For this review, take the finished solid that the model builds, in its own axes (mm). Face numbers are marked on the shaded views. A direction names the side the tool comes from. Give positions to 0.01 mm unless a question says otherwise; leave off trailing zeros. Loops run counter-clockwise (first coordinate to the right, second up) from the corner with the lowest first, then second, coordinate; pieces in that order, holes last. Notation, with made-up numbers: (-9.5, -37.5) - (0.5, -37.5) arc R23 ccw to (0.5, -6.5) - close; hole circle Ø9 at (11.5, 10.25). An arc over 180 degrees is marked (long way). Answer as CSV lines item,"result".
from build123d import *

# Parameters (mm, degrees)
SKETCH3_W           = 52
SKETCH3_H           = 52
BOSS_EXTRUDE1_DEPTH = 10
SKETCH4_R           = 2
CUT_EXTRUDE1_DEPTH  = 10
SKETCH5_R           = 25
CUT_EXTRUDE2_DEPTH  = 3
SKETCH6_R           = 16
CUT_EXTRUDE3_DEPTH  = 38.429934544
SKETCH8_W           = 21.53152206
SKETCH8_H           = 52
BOSS_EXTRUDE2_DEPTH = 52
SKETCH9_R           = 20
CUT_EXTRUDE4_DEPTH  = 21.53152206
BOSS_EXTRUDE3_DEPTH = 52
SKETCH11_R          = 20
CUT_EXTRUDE5_DEPTH  = 52
SKETCH12_W          = 34.659031173
SKETCH12_H          = 60
CUT_EXTRUDE6_DEPTH  = 10


with BuildPart() as part:
    # Sketch3 → Boss-Extrude1 (new body)
    with BuildSketch(Plane.XY):
        Rectangle(SKETCH3_W, SKETCH3_H)
    extrude(amount=BOSS_EXTRUDE1_DEPTH)

    # Sketch4 → Cut-Extrude1 (cut)
    with BuildSketch(Plane(origin=(0, 0, 0), x_dir=(-1, 0, 0), z_dir=(0, 0, -1))):
        with Locations((-21, 21)):
            Circle(SKETCH4_R)
        with Locations(Location((21, 21, 0), (0, 0, 180))):
            Circle(SKETCH4_R)
        with Locations((21, -21)):
            Circle(SKETCH4_R)
        with Locations(Location((-21, -21, 0), (0, 0, 180))):
            Circle(SKETCH4_R)
    extrude(amount=-CUT_EXTRUDE1_DEPTH, mode=Mode.SUBTRACT)

    # Sketch5 → Cut-Extrude2 (cut)
    with BuildSketch(Plane(origin=(0, 0, 0), x_dir=(-1, 0, 0), z_dir=(0, 0, -1))):
        Circle(SKETCH5_R)
    extrude(amount=-CUT_EXTRUDE2_DEPTH, mode=Mode.SUBTRACT)

    # Sketch6 → Cut-Extrude3 (cut, through all)
    with BuildSketch(Plane(origin=(0, 0, 3), x_dir=(-1, 0, 0), z_dir=(0, 0, -1))):
        Circle(SKETCH6_R)
    extrude(amount=-CUT_EXTRUDE3_DEPTH, mode=Mode.SUBTRACT)

    # Sketch8 → Boss-Extrude2 (add)
    with BuildSketch(Plane.ZY.offset(26)):
        with Locations((20.76576103, 0)):
            Rectangle(SKETCH8_W, SKETCH8_H)
    extrude(amount=-BOSS_EXTRUDE2_DEPTH)

    # Sketch9 → Cut-Extrude4 (cut)
    with BuildSketch(Plane.XY.offset(31.53152206)):
        Circle(SKETCH9_R)
    extrude(amount=-CUT_EXTRUDE4_DEPTH, mode=Mode.SUBTRACT)

    # Sketch10 → Boss-Extrude3 (add)
    with BuildSketch(Plane.ZY.offset(26)):
        with BuildLine():
            Line((31.53152206, 26), (31.53152206, -26))
            ThreePointArc((31.53152206, -26), (57.53152206, 0), (31.53152206, 26))
        make_face()
    extrude(amount=-BOSS_EXTRUDE3_DEPTH)

    # Sketch11 → Cut-Extrude5 (cut)
    with BuildSketch(Plane.ZY.offset(26)):
        with Locations(Location((31.53152206, 0, 0), (0, 0, 270))):
            Circle(SKETCH11_R)
    extrude(amount=-CUT_EXTRUDE5_DEPTH, mode=Mode.SUBTRACT)

    # Sketch12 → Cut-Extrude6 (cut)
    with BuildSketch(Plane(origin=(22, 0, 0), x_dir=(0, 0, -1), z_dir=(1, 0, 0))):
        with Locations((-41.329515587, 0)):
            Rectangle(SKETCH12_W, SKETCH12_H)
    extrude(amount=-CUT_EXTRUDE6_DEPTH, mode=Mode.SUBTRACT)


solid = part.part
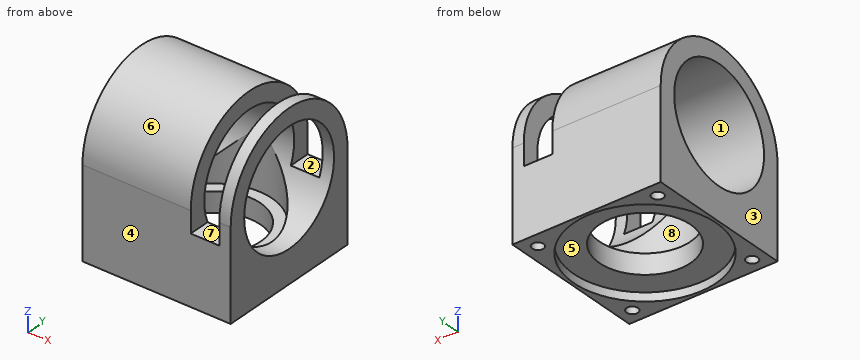
1) Consider section B-B on x = 0. Write out the cut boundary in (y, z), and give its area (3 significant figures).
From the geometry:
outline,"(-26, 0) - (-25, 0) - (-25, 3) - (-16, 3) - (-16, 10) - (-20, 10) - (-20, 31.53) arc R20 cw to (20, 31.53) - (20, 10) - (16, 10) - (16, 3) - (25, 3) - (25, 0) - (26, 0) - (26, 31.53) arc R26 ccw to (-26, 31.53) - close"
area,"838 mm^2"
2) Wall thickness on line 1 (Y direction, x = -21, z = 7); line 2 (X direction, y = 3, z = 52); line 3 (Y direction, x = 0, z = 20.5): over which ranges is each line inside the solid? List them lowest first. Write a range as from..to.
From the geometry:
line 1,"y = -26..-23, -19..19, 23..26"
line 2,"x = -26..12, 22..26"
line 3,"y = -26..-20, 20..26"
3) Insertion check: P1, Ø1.5, axis at x = 9.5, y = 3, coming from the +Z side; P2, Ø10, axis at y = -10, z = 29, coming from the -X side; P3, Ø4, axis at x = 12, z = 46, coming from the -Y side; P4, Ø10, axis at x = 18, y = -11.5, coming from the +Z side. Each pin has a flat end and moves straight along its axis. Give the tip position at first contact, or say it passes through.
From the geometry:
P1,"stops at z = 57.43"
P2,"passes through"
P3,"stops at y = -22.82"
P4,"stops at z = 56.1"
4) Draft analysis for pull direction Z (two halves, no side actions). For the marked faces 1, 2 and 3, state which applies: pulls with the +Z half, pulls with the -Z half, needs draft (parallel to the pull), parting line crosses it, or undercut.
From the geometry:
face 1,"undercut"
face 2,"pulls with the +Z half"
face 3,"needs draft"
5) Machinability: for the marked faces 4, 5, 6, 7 and 8, which of the approach directions +Z, -Z, +X, -X, +Y, -Y give a long, thin tool a straight path to every point of the face, cutting with its end or side? Answer none if there is none.
From the geometry:
face 4,"+Z, -Z, +X, -X, -Y"
face 5,"-Z"
face 6,"+Z, +X, -X"
face 7,"+Z, +Y, -Y"
face 8,"none"
6) Consider section D-D on z = 33. Write out the cut boundary in (x, y).
From the geometry:
outline,"(-26, -25.96) - (12, -25.96) - (12, -19.95) - (-26, -19.95) - close; (-26, 19.95) - (12, 19.95) - (12, 25.96) - (-26, 25.96) - close; (22, -25.96) - (26, -25.96) - (26, -19.95) - (22, -19.95) - close; (22, 19.95) - (26, 19.95) - (26, 25.96) - (22, 25.96) - close"
7) Consider section C-C on x = -21. Write out the cut boundary in (y, z), and give its area (3 significant figures).
From the geometry:
outline,"(-26, 0) - (-23, 0) - (-23, 10) - (-19, 10) - (-19, 0) - (-13.56, 0) - (-13.56, 3) - (13.56, 3) - (13.56, 0) - (19, 0) - (19, 10) - (23, 10) - (23, 0) - (26, 0) - (26, 31.53) arc R26 ccw to (-26, 31.53) - close; hole circle Ø40 at (0, 31.53)"
area,"1,280 mm^2"
8) Consider section A-A on y = 0. Write out the cut boundary in (x, z), and give its area (3 significant figures).
From the geometry:
outline,"(-26, 0) - (-25, 0) - (-25, 3) - (-16, 3) - (-16, 10) - (-20, 10) - (-20, 11.53) - (-26, 11.53) - close; (-26, 51.53) - (12, 51.53) - (12, 57.53) - (-26, 57.53) - close; (16, 3) - (25, 3) - (25, 0) - (26, 0) - (26, 11.53) - (20, 11.53) - (20, 10) - (16, 10) - close; (22, 51.53) - (26, 51.53) - (26, 57.53) - (22, 57.53) - close"
area,"416 mm^2"
